from build123d import *

# Parameters (mm, degrees)
SKETCH1_W                       = 470
SKETCH1_H                       = 260
BOSS_EXTRUDE1_DEPTH             = 12.5
SKETCH4_W                       = 70
SKETCH4_H                       = 97
CUT_EXTRUDE3_DEPTH              = 97
SKETCH5_R                       = 2.75
CUT_EXTRUDE4_DEPTH              = 97
SKETCH6_R                       = 5
CUT_EXTRUDE5_DEPTH              = 8
SKETCH7_W                       = 593.529724836
SKETCH7_H                       = 137.698896162
CUT_EXTRUDE6_DEPTH              = 40
M8_TAPPED_HOLE1_D               = 6.8
M8_TAPPED_HOLE1_DEPTH           = 20
M8_TAPPED_HOLE1_TIP             = 2.042926105
M10_TAPPED_HOLE1_D              = 8.5
M10_TAPPED_HOLE1_DEPTH          = 27.5
M10_TAPPED_HOLE1_TIP            = 2.553657631
SKETCH13_R                      = 19
CUT_EXTRUDE7_DEPTH              = 270.722079185
SKETCH14_R                      = 21
CUT_EXTRUDE8_DEPTH              = 12
LPATTERN1_COUNT                 = 3
LPATTERN1_PITCH                 = 90
SKETCH15_R                      = 3.25
CUT_EXTRUDE9_DEPTH              = 270.722079185
SKETCH16_R                      = 5.5
CUT_EXTRUDE10_DEPTH             = 10
LPATTERN2_COUNT                 = 2
LPATTERN2_PITCH                 = 447
M6_TAPPED_HOLE1_D               = 5
M6_TAPPED_HOLE1_DEPTH           = 14.5
M6_TAPPED_HOLE1_TIP             = 1.502151548
M6_TAPPED_HOLE1_ON_FACE_2_D     = 5
M6_TAPPED_HOLE1_ON_FACE_2_DEPTH = 14.5
M6_TAPPED_HOLE1_ON_FACE_2_TIP   = 1.502151548


with BuildPart() as part:
    # Sketch1 → Boss-Extrude1 (new, symmetric)
    with BuildSketch(Plane.XY):
        Rectangle(SKETCH1_W, SKETCH1_H)
    extrude(amount=BOSS_EXTRUDE1_DEPTH, both=True)

    # Sketch4 → Cut-Extrude3 (cut)
    with BuildSketch(Plane.XY.offset(12.5)):
        with Locations((-170, 81.5)):
            Rectangle(SKETCH4_W, SKETCH4_H)
        with Locations((-80, 81.5)):
            Rectangle(SKETCH4_W, SKETCH4_H)
        with Locations((10, 81.5)):
            Rectangle(SKETCH4_W, SKETCH4_H)
        with Locations((180, 81.5)):
            Rectangle(SKETCH4_W, SKETCH4_H)
    extrude(amount=-CUT_EXTRUDE3_DEPTH, mode=Mode.SUBTRACT)

    # Sketch5 → Cut-Extrude4 (cut)
    with BuildSketch(Plane.XY.offset(12.5)):
        with Locations((115, 19.25)):
            Circle(SKETCH5_R)
    extrude(amount=-CUT_EXTRUDE4_DEPTH, mode=Mode.SUBTRACT)

    # Sketch6 → Cut-Extrude5 (cut)
    with BuildSketch(Plane(origin=(0, 0, -12.5), x_dir=(-1, 0, 0), z_dir=(0, 0, -1))):
        with Locations((-115, 19.25)):
            Circle(SKETCH6_R)
    extrude(amount=-CUT_EXTRUDE5_DEPTH, mode=Mode.SUBTRACT)

    # Sketch7 → Cut-Extrude6 (cut)
    with BuildSketch(Plane(origin=(0, 0, -12.5), x_dir=(-1, 0, 0), z_dir=(0, 0, -1))):
        with Locations((25.503124985, -158.849448081)):
            Rectangle(SKETCH7_W, SKETCH7_H)
    extrude(amount=-CUT_EXTRUDE6_DEPTH, mode=Mode.SUBTRACT)

    # M8 Tapped Hole1
    with Locations(Plane(origin=(0, 130, 0), x_dir=(1, 0, 0), z_dir=(0, 1, 0))):
        with Locations((-220, 0), (225, 0), (135, 0), (-35, 0), (-125, 0), (60, 0)):
            Hole(M8_TAPPED_HOLE1_D / 2, depth=M8_TAPPED_HOLE1_DEPTH)
            with Locations((0, 0, -(M8_TAPPED_HOLE1_DEPTH + M8_TAPPED_HOLE1_TIP / 2))):  # 118° drill point
                Cone(0, M8_TAPPED_HOLE1_D / 2, M8_TAPPED_HOLE1_TIP, mode=Mode.SUBTRACT)

    # M10 Tapped Hole1
    with Locations(Plane(origin=(0, -90, 0), x_dir=(-1, 0, 0), z_dir=(0, -1, 0))):
        with Locations((-155, 0), (155, 0)):
            Hole(M10_TAPPED_HOLE1_D / 2, depth=M10_TAPPED_HOLE1_DEPTH)
            with Locations((0, 0, -(M10_TAPPED_HOLE1_DEPTH + M10_TAPPED_HOLE1_TIP / 2))):  # 118° drill point
                Cone(0, M10_TAPPED_HOLE1_D / 2, M10_TAPPED_HOLE1_TIP, mode=Mode.SUBTRACT)

    # Sketch13 → Cut-Extrude7 (cut, through all)
    with BuildSketch(Plane.XY.offset(12.5)):
        with Locations((-170, 6)):
            Circle(SKETCH13_R)
    cut_extrude7 = extrude(amount=-CUT_EXTRUDE7_DEPTH, mode=Mode.SUBTRACT)

    # Sketch14 → Cut-Extrude8 (cut)
    with BuildSketch(Plane.XY.offset(12.5)):
        with Locations((-170, 6)):
            Circle(SKETCH14_R)
    cut_extrude8 = extrude(amount=-CUT_EXTRUDE8_DEPTH, mode=Mode.SUBTRACT)

    # LPattern1: Cut-Extrude7, Cut-Extrude8 ×3
    with Locations(*[(i * LPATTERN1_PITCH, 0, 0) for i in range(1, LPATTERN1_COUNT)]):
        add(cut_extrude7, mode=Mode.SUBTRACT)
        add(cut_extrude8, mode=Mode.SUBTRACT)

    # Sketch15 → Cut-Extrude9 (cut, through all)
    with BuildSketch(Plane(origin=(0, 0, -12.5), x_dir=(-1, 0, 0), z_dir=(0, 0, -1))):
        with Locations((-227, 90)):
            Circle(SKETCH15_R)
        with Locations((-227, -50)):
            Circle(SKETCH15_R)
    cut_extrude9 = extrude(amount=-CUT_EXTRUDE9_DEPTH, mode=Mode.SUBTRACT)

    # Sketch16 → Cut-Extrude10 (cut)
    with BuildSketch(Plane(origin=(0, 0, -12.5), x_dir=(-1, 0, 0), z_dir=(0, 0, -1))):
        with Locations((-227, 90)):
            Circle(SKETCH16_R)
        with Locations((-227, -50)):
            Circle(SKETCH16_R)
    cut_extrude10 = extrude(amount=-CUT_EXTRUDE10_DEPTH, mode=Mode.SUBTRACT)

    # LPattern2: Cut-Extrude9, Cut-Extrude10 ×2
    with Locations(*[(-i * LPATTERN2_PITCH, 0, 0) for i in range(1, LPATTERN2_COUNT)]):
        add(cut_extrude9, mode=Mode.SUBTRACT)
        add(cut_extrude10, mode=Mode.SUBTRACT)

    # M6 Tapped Hole1
    with Locations(Plane(origin=(-235, 20, 0), x_dir=(0, 0, -1), z_dir=(-1, 0, 0))):
        with Locations((0, 0)):
            Hole(M6_TAPPED_HOLE1_D / 2, depth=M6_TAPPED_HOLE1_DEPTH)
            with Locations((0, 0, -(M6_TAPPED_HOLE1_DEPTH + M6_TAPPED_HOLE1_TIP / 2))):  # 118° drill point
                Cone(0, M6_TAPPED_HOLE1_D / 2, M6_TAPPED_HOLE1_TIP, mode=Mode.SUBTRACT)

    # M6 Tapped Hole1 on face 2
    with Locations(Plane(origin=(235, 20, 0), x_dir=(0, 0, 1), z_dir=(1, 0, 0))):
        with Locations((0, 0)):
            Hole(M6_TAPPED_HOLE1_ON_FACE_2_D / 2, depth=M6_TAPPED_HOLE1_ON_FACE_2_DEPTH)
            with Locations((0, 0, -(M6_TAPPED_HOLE1_ON_FACE_2_DEPTH + M6_TAPPED_HOLE1_ON_FACE_2_TIP / 2))):  # 118° drill point
                Cone(0, M6_TAPPED_HOLE1_ON_FACE_2_D / 2, M6_TAPPED_HOLE1_ON_FACE_2_TIP, mode=Mode.SUBTRACT)


solid = part.part
Check sheet for the modelled part. Datum: model origin and axes. Units: mm. A direction names the side the tool comes from. Give positions to 0.01 mm unless a question says otherwise; leave off trailing zeros. Loops run counter-clockwise (first coordinate to the right, second up) from the corner with the lowest first, then second, coordinate; pieces in that order, holes last. Notation, with made-up numbers: M 27.25,-17.5 L 73.25,-17.5 A27 cw 73.25,9.5 Z; hole C 22,52 d5. An arc over 180 degrees is marked long. Use a Markdown table: item, result. Add a question column.
Q1. Go/stop test with flat-tipped pins: pin 1 (2 mm diameter, centred on x = -55, z = 0.5, fed in from +Y); pin 2 (9 mm diameter, centred on x = -218.5, y = 90.5, fed in from -Z); pin 3 (4 mm diameter, centred on x = -220, z = 0, fed in from +Y); pin 4 (7.5 mm diameter, centred on x = 227, y = 90, fed in from -Z). Record where each tip stops, or that it passes through.
Q2. Scan lines: line 1 along X through (y, z) = (65.5, -8.5); line 2 along Y through (x, z) = (-220, -10.5); line 3 along Z through (x, y) = (-125, 124.5). Record each from-to range of solid material in increasing order. Write a range as [from, to].
Q3. Sectioned sample at B-B, the plane x = -80. Record the cut outline in (y, z), then the cut area to 3 significant figures.
Q4. Tool access check on faces 5 (the cylindrical face through (28.12, 11.71, -5.91)), 6 (the cylindrical face through (150.754, -76.057, -0.187)), 7 (the cylindrical face through (-214.505, -49.758, -7.57)), 8 (the flat face through (-135, 81, 0)). Record the directions out of +Z, -Z, +X, -X, +Y, -Y that give a thin tool (end or side, any length) a straight path to the whole face; none if there is none.
Q5. Sectioned sample at D-D, the plane x = 192. Record the cut outline in (y, z).
Q6. Sectioned sample at A-A, the plane y = 116. Give the number of separate pieces and of enclosed holes in the cut face, then the cut area to 3 significant figures.
Q7. Mould release check, pull along Y, two halves, no side actions. Record for faces 1 (the flat face through (-3, -27, -12.5)), 2 (the flat face through (-6, -5, 0.5)), 3 (the conical face through (-154.26, -60.39, -0.03)), 4 (the cylindrical face through (-215.95, 93.72, -7.57)): pulls with the +Y half, pulls with the -Y half, needs draft (parallel to the pull), parting line crosses it, or undercut.
Verdict:
| question | item | result |
|---|---|---|
| 1 | pin 1 | y = 33 |
| 1 | pin 2 | z = -12.5 |
| 1 | pin 3 | y = 109.16 |
| 1 | pin 4 | z = -2.5 |
| 2 | line 1 | [-235, -205], [-135, -115], [-45, -25], [45, 145], [215, 235] |
| 2 | line 2 | [-90, -55.5], [-44.5, 84.5], [95.5, 130] |
| 2 | line 3 | [-12.5, -3.4], [3.4, 12.5] |
| 3 | outline | M -90,-12.5 L -13,-12.5 L -13,0.5 L -15,0.5 L -15,12.5 L -90,12.5 Z; M 25,-12.5 L 33,-12.5 L 33,12.5 L 27,12.5 L 27,0.5 L 25,0.5 Z |
| 3 | area | 2,080 mm^2 |
| 4 | face 5 | +Z, -Z |
| 4 | face 6 | -Y |
| 4 | face 7 | -Z |
| 4 | face 8 | +Z, -Z, +Y |
| 5 | outline | M -90,-12.5 L 33,-12.5 L 33,12.5 L -90,12.5 Z |
| 6 | separate pieces | 5 |
| 6 | enclosed holes | 6 |
| 6 | area | 4,530 mm^2 |
| 7 | face 1 | needs draft |
| 7 | face 2 | undercut |
| 7 | face 3 | pulls with the -Y half |
| 7 | face 4 | undercut |
